Print and shaded views of the part. All mm, measured from the part's lowest x, y and z. Round coordinates to 2 decimals unless told otherwise and drop trailing zeros. Loops run counter-clockwise (first coordinate to the right, second up) from the corner with the lowest first, then second, coordinate; pieces in that order, holes last. Notation, with made-up numbers: (-24.5, 3.5) -> (8.5, 3.5) arc R24 ccw to (8.5, 28.5) -> close; hole circle Ø8 at (14, 22.5). An arc over 180 degrees is marked (long way). Answer as CSV lines item,"result".
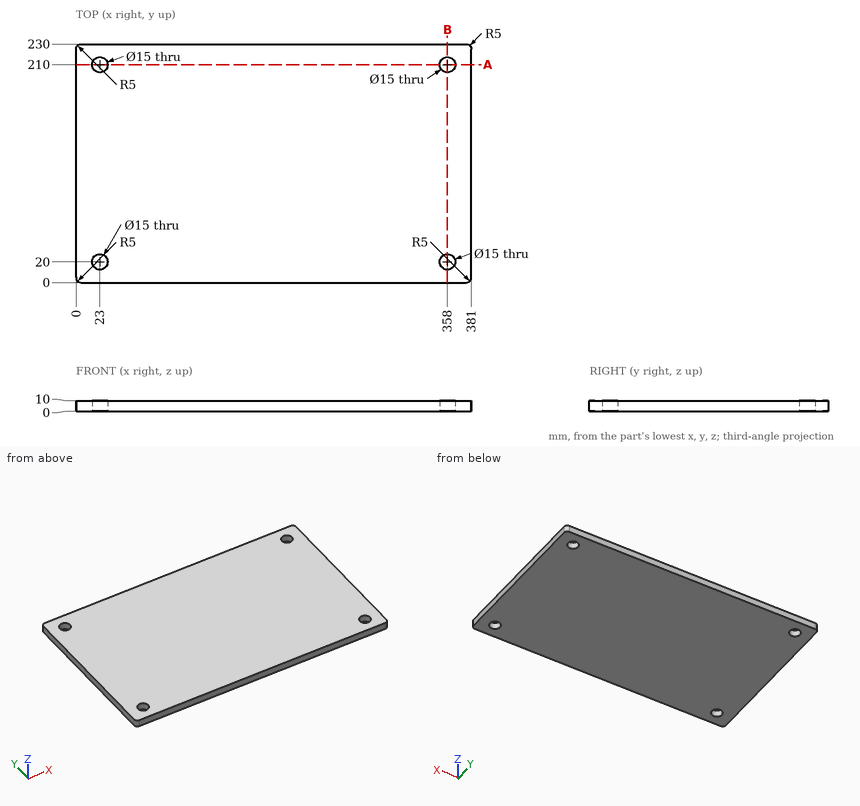
Q1. Probe L1, parallel to Y at x = 23, z = 6; L2, parallel to X at y = 24, z = 1; L3, parallel to X at y = 26, z = 5.5. List the from-to ranges inside material, lowest first. Write a range as [from, to].
Results:
L1,"[0, 12.5], [27.5, 202.5], [217.5, 230]"
L2,"[0, 16.66], [29.34, 351.66], [364.34, 381]"
L3,"[0, 18.5], [27.5, 353.5], [362.5, 381]"
Q2. Slice it at A-A, the plane y = 210. Give the cut face in (x, z).
Results:
outline,"(0, 0) -> (15.5, 0) -> (15.5, 10) -> (0, 10) -> close; (30.5, 0) -> (350.5, 0) -> (350.5, 10) -> (30.5, 10) -> close; (365.5, 0) -> (381, 0) -> (381, 10) -> (365.5, 10) -> close"
Q3. Slice it at B-B, the plane x = 358. Give the cut face in (y, z).
Results:
outline,"(0, 0) -> (12.5, 0) -> (12.5, 10) -> (0, 10) -> close; (27.5, 0) -> (202.5, 0) -> (202.5, 10) -> (27.5, 10) -> close; (217.5, 0) -> (230, 0) -> (230, 10) -> (217.5, 10) -> close"
